Geometry: final body of the model. Coordinates: model frame, mm. A direction names the side the tool comes from. Give positions to 0.01 mm unless a question says otherwise; leave off trailing zeros. Loops run counter-clockwise (first coordinate to the right, second up) from the corner with the lowest first, then second, coordinate; pieces in that order, holes last. Notation, with made-up numbers: (-5.5, -32.75) -> (7.5, -32.75) arc R22 ccw to (7.5, 4.25) -> close; hole circle Ø11 at (27, 14). An arc over 180 degrees is marked (long way). Answer in a Markdown table with one row per item. Add a question column.
1) Draft query along Y for faces 1 (the flat face through (5, -2, -101.14)), 2 (the cylindrical face through (-3.65, -4.76, 104.9)), 3 (the cylindrical face through (0.07, 0.751, -110.385)). Return one class per face: +Y half, -Y half, draft (parallel to the pull), parting line (faces both ways), or undercut.
2) Section query B-B (x = 0). Give the number of separate pieces and of enclosed holes in the cut face, plus the area to 3 significant figures.
3) Line query: line 1 (Z direction, x = -4.5, y = 2.75); line 2 (Z direction, x = 0.5, y = 5.75); line 3 (Y direction, x = -0.5, z = -108). Output: solid intervals per line, ascending. Write a range as from..to.
4) First-contact query: P1, Ø0.8, axis at x = -5.5, y = -0.5, coming from the -Z side; P2, Ø5.5, axis at x = 1.5, z = -106, coming from the -Y side; P3, Ø3.5, axis at y = 0.5, z = 109, coming from the +X side. Flat tips, straight axial feed; report the tip coordinate or a pass-through.
5) Access query for faces 4 (the flat face through (0, -5, -108)), 5 (the flat face through (-5, 2, -106)), 6 (the flat face through (5, 2, 106)), 7 (the flat face through (-4, 3, 101.14)). Directions: +Z, -Z, +X, -X, +Y, -Y. A direction counts if a zero-diameter tool reaches every point of the face in a straight line with its end or side. Return the directions, or none.
6) Section query D-D (z = -59). Return the cut outline in (x, y), plus the area to 3 significant figures.
7) Section query A-A (z = 108). Return the cut outline in (x, y), plus the area to 3 significant figures.
```python
from build123d import *

# Parameters (mm, degrees)
SKETCH_1_R          = 6
EXTRUDE_1_DEPTH     = 113
SKETCH_2_W          = 1.14
SKETCH_2_H          = 0.9
SKETCH_2_H_2        = 1.654271951
CUT_EXTRUDE_START   = -10
CUT_EXTRUDE_1_DEPTH = 10
HOLE_WIZARD_M6_1_D  = 5


with BuildPart() as part:
    # 草图1 → 凸台-拉伸1 (new, symmetric)
    with BuildSketch(Plane.XY):
        Circle(SKETCH_1_R)
    extrude(amount=EXTRUDE_1_DEPTH, both=True)

    # 草图2 → 切除-旋转1 (revolve, cut)
    with BuildSketch(Plane(origin=(0, 0, 0), x_dir=(0, 0, -1), z_dir=(1, 0, 0)), mode=Mode.PRIVATE) as cut_revolve_1_sk:
        with Locations((100.57, 5.55)):
            Rectangle(SKETCH_2_W, SKETCH_2_H)
        with Locations((-100.57, 5.172864024)):
            Rectangle(SKETCH_2_W, SKETCH_2_H_2)
    revolve(cut_revolve_1_sk.sketch.rotate(Axis((0, 0, 0), (0, 0, -1)), 180), axis=Axis((0, 0, 0), (0, 0, -1)), mode=Mode.SUBTRACT)

    # 草图3 → 切除-拉伸1 (cut)
    with BuildSketch(Plane(origin=(0, 0, -113), x_dir=(-1, 0, 0), z_dir=(0, 0, -1)).offset(CUT_EXTRUDE_START)):
        with BuildLine():
            Line((-5, 3.31662479), (-5, -3.31662479))
            ThreePointArc((-5, -3.31662479), (-6, 0), (-5, 3.31662479))
        make_face()
        with BuildLine():
            Line((5, 3.31662479), (5, -3.31662479))
            ThreePointArc((5, -3.31662479), (6, 0), (5, 3.31662479))
        make_face()
        with BuildLine():
            Line((-3.31662479, 5), (3.31662479, 5))
            ThreePointArc((3.31662479, 5), (0, 6), (-3.31662479, 5))
        make_face()
        with BuildLine():
            Line((3.31662479, -5), (-3.31662479, -5))
            ThreePointArc((-3.31662479, -5), (0, -6), (3.31662479, -5))
        make_face()
    cut_extrude_1 = extrude(amount=CUT_EXTRUDE_1_DEPTH, mode=Mode.SUBTRACT)

    # M6 螺纹孔1 (through all)
    with Locations(Plane.ZY.offset(5)):
        with Locations((-108, 0)):
            hole_wizard_m6_1 = Hole(HOLE_WIZARD_M6_1_D / 2)

    # 镜向1: 切除-拉伸1, M6 螺纹孔1 across plane
    add(cut_extrude_1.mirror(Plane.XY), mode=Mode.SUBTRACT)
    add(hole_wizard_m6_1.mirror(Plane.XY), mode=Mode.SUBTRACT)


solid = part.part
```
Evaluation:
| question | item | result |
|---|---|---|
| 1 | face 1 | draft |
| 1 | face 2 | parting line |
| 1 | face 3 | undercut |
| 2 | separate pieces | 1 |
| 2 | enclosed holes | 2 |
| 2 | area | 2,630 mm² |
| 3 | line 1 | -113..-101.14, -100..100, 101.14..113 |
| 3 | line 2 | -103..-101.14, -100..100, 101.14..103 |
| 3 | line 3 | -5..-2.5, 2.5..5 |
| 4 | P1 | z = -103 |
| 4 | P2 | y = -5 |
| 4 | P3 | x = 5 |
| 5 | face 4 | -Z, +X, -X, -Y |
| 5 | face 5 | -Z, -X, +Y, -Y |
| 5 | face 6 | +Z, +X, +Y, -Y |
| 5 | face 7 | none |
| 6 | outline | circle Ø12 at (0, 0) |
| 6 | area | 113 mm² |
| 7 | outline | (-5, -3.32) arc R6 ccw to (-3.32, -5) -> (3.32, -5) arc R6 ccw to (5, -3.32) -> (5, -2.5) -> (-5, -2.5) -> close; (-5, 2.5) -> (5, 2.5) -> (5, 3.32) arc R6 ccw to (3.32, 5) -> (-3.32, 5) arc R6 ccw to (-5, 3.32) -> close |
| 7 | area | 45.1 mm² |
